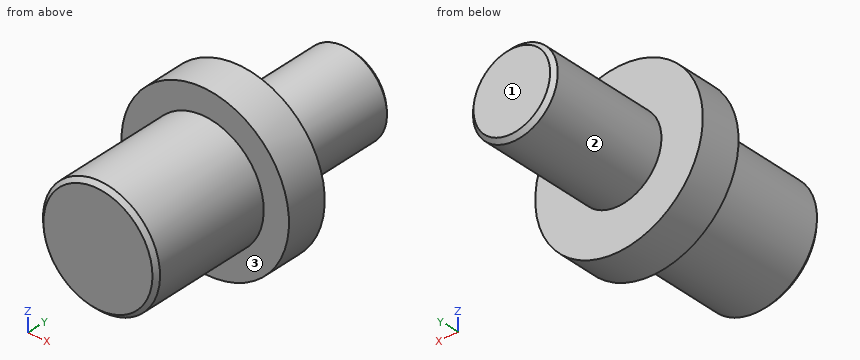
```python
from build123d import *

# Parameters (mm, degrees)
CHAMFER1_SIZE = 0.2


with BuildPart() as part:
    # Sketch1 → Revolve1 (revolve)
    with BuildSketch(Plane.XY, mode=Mode.PRIVATE) as revolve1_sk:
        Polygon((0, 0), (0, 14), (2.1, 14), (2.1, 8), (4.15, 8), (4.15, 6), (2.9, 6), (2.9, 0), align=None)
    revolve(revolve1_sk.sketch.rotate(Axis((0, 0, 0), (0, 1, 0)), 90), axis=Axis((0, 0, 0), (0, 1, 0)))

    # Chamfer1
    chamfer1_edges = [part.edges().sort_by_distance(p)[0] for p in [
        (0, 14, 2.1),
        (0, 0, 2.9),
    ]]
    chamfer(chamfer1_edges, length=CHAMFER1_SIZE)


solid = part.part
```
The listing builds one solid part. Answer for the finished solid, in the listing's coordinates (mm). Face numbers are marked on the shaded views. A direction names the side the tool comes from. Give positions to 0.01 mm unless a question says otherwise; leave off trailing zeros. Write each loop counter-clockwise with the first axis right and the second up, starting at its lowest first coordinate (ties: lowest second). Pieces come first, ordered by that corner, then holes. Notation, with made-up numbers: (48.25, -7) -> (72.25, -7) arc R14 ccw to (72.25, 20) -> close; hole circle Ø9 at (29.5, -15). An arc over 180 degrees is marked (long way). Use one line per item in the form item = value.
1) Section B-B on z = 0 is taken. Write down the section's boundary in (x, y).
Result:
outline = (-4.15, 6) -> (-2.9, 6) -> (-2.9, 0.2) -> (-2.7, 0) -> (2.7, 0) -> (2.9, 0.2) -> (2.9, 6) -> (4.15, 6) -> (4.15, 8) -> (2.1, 8) -> (2.1, 13.8) -> (1.9, 14) -> (-1.9, 14) -> (-2.1, 13.8) -> (-2.1, 8) -> (-4.15, 8) -> close
2) Section A-A on x = 0 is taken. Write down the section's boundary in (y, z).
Result:
outline = (0, -2.7) -> (0.2, -2.9) -> (6, -2.9) -> (6, -4.15) -> (8, -4.15) -> (8, -2.1) -> (13.8, -2.1) -> (14, -1.9) -> (14, 1.9) -> (13.8, 2.1) -> (8, 2.1) -> (8, 4.15) -> (6, 4.15) -> (6, 2.9) -> (0.2, 2.9) -> (0, 2.7) -> close
3) Section D-D on y = 9.5 is taken. Write down the section's boundary in (x, z).
Result:
outline = circle Ø4.2 at (0, 0)
4) Section C-C on y = 3.5 is taken. Write down the section's boundary in (x, z), plus the area to 3 significant figures.
Result:
outline = circle Ø5.8 at (0, 0)
area = 26.4 mm²
5) A tool of negligible diameter and unlimited length cuts with its end or side. For the marked faces 1, 2 and 3, from which of +Z, -Z, +X, -X, +Y, -Y can it reach the whole face along a straight path? Write none if from no direction.
Result:
face_1 = +Z, -Z, +X, -X, +Y
face_2 = +Y
face_3 = -Y
6) Each of these flat-tipped pins is pushed along its axis until it touches: P1, Ø1, axis at x = 1, y = 7.5, coming from the +Z side; P2, Ø1.5, axis at y = 12.5, z = 2, coming from the -X side; P3, Ø2, axis at y = 10, z = 2.5, coming from the +X side. Where does it stop, or does it pass through?
Result:
P1 = 4.12
P2 = -1.69
P3 = 1.47
7) Straight lines are drawn through the part: probe 1 along Y at (x, z) = (2.25, -3); probe 2 along Y at (x, z) = (2, -0.75); probe 3 along Z at (x, y) = (-1, 0.5). For each, find the intervals that lie inside material, in ascending order.
Result:
probe_1 = 6 to 8
probe_2 = 0 to 8
probe_3 = -2.72 to 2.72
